```python
from build123d import *

# Parameters (mm, degrees)
SKETCH1_W           = 36
SKETCH1_H           = 55
BOSS_EXTRUDE1_DEPTH = 4
SKETCH2_R           = 1.5
CUT_EXTRUDE1_DEPTH  = 4
FILLET1_R           = 1.5
BOSS_EXTRUDE2_DEPTH = 4


with BuildPart() as part:
    # Sketch1 → Boss-Extrude1 (new body)
    with BuildSketch(Plane.XY):
        Rectangle(SKETCH1_W, SKETCH1_H)
    extrude(amount=BOSS_EXTRUDE1_DEPTH)

    # Sketch2 → Cut-Extrude1 (cut)
    with BuildSketch(Plane.XY.offset(4)):
        with BuildLine():
            Line((-14.75, 23), (-12, 23))
            ThreePointArc((-12, 23), (-10.5, 24.5), (-12, 26))
            Line((-12, 26), (-14.75, 26))
            ThreePointArc((-14.75, 26), (-16.25, 24.5), (-14.75, 23))
        make_face()
        with BuildLine():
            Line((12, 23), (14.75, 23))
            ThreePointArc((14.75, 23), (16.25, 24.5), (14.75, 26))
            Line((14.75, 26), (12, 26))
            ThreePointArc((12, 26), (10.5, 24.5), (12, 23))
        make_face()
        with BuildLine():
            Line((-8, 4), (-7, 4))
            ThreePointArc((-7, 4), (-5.5, 5.5), (-7, 7))
            Line((-7, 7), (-8, 7))
            ThreePointArc((-8, 7), (-9.5, 5.5), (-8, 4))
        make_face()
        with Locations((-2, 5.5)):
            Circle(SKETCH2_R)
        with Locations((2, 5.5)):
            Circle(SKETCH2_R)
        with BuildLine():
            Line((7, 4), (8, 4))
            ThreePointArc((8, 4), (9.5, 5.5), (8, 7))
            Line((8, 7), (7, 7))
            ThreePointArc((7, 7), (5.5, 5.5), (7, 4))
        make_face()
        with BuildLine():
            Line((7, -6), (8, -6))
            ThreePointArc((8, -6), (9.5, -4.5), (8, -3))
            Line((8, -3), (7, -3))
            ThreePointArc((7, -3), (5.5, -4.5), (7, -6))
        make_face()
        with Locations((2, -4.5)):
            Circle(SKETCH2_R)
        with Locations((-2, -4.5)):
            Circle(SKETCH2_R)
        with BuildLine():
            Line((-8, -6), (-7, -6))
            ThreePointArc((-7, -6), (-5.5, -4.5), (-7, -3))
            Line((-7, -3), (-8, -3))
            ThreePointArc((-8, -3), (-9.5, -4.5), (-8, -6))
        make_face()
        with BuildLine():
            Line((-8, -16), (-7, -16))
            ThreePointArc((-7, -16), (-5.5, -14.5), (-7, -13))
            Line((-7, -13), (-8, -13))
            ThreePointArc((-8, -13), (-9.5, -14.5), (-8, -16))
        make_face()
        with BuildLine():
            Line((-8, -26), (-7, -26))
            ThreePointArc((-7, -26), (-5.5, -24.5), (-7, -23))
            Line((-7, -23), (-8, -23))
            ThreePointArc((-8, -23), (-9.5, -24.5), (-8, -26))
        make_face()
        with Locations((-2, -14.5)):
            Circle(SKETCH2_R)
        with Locations((-2, -24.5)):
            Circle(SKETCH2_R)
        with Locations((2, -14.5)):
            Circle(SKETCH2_R)
        with Locations((2, -24.5)):
            Circle(SKETCH2_R)
        with BuildLine():
            Line((7, -26), (8, -26))
            ThreePointArc((8, -26), (9.5, -24.5), (8, -23))
            Line((8, -23), (7, -23))
            ThreePointArc((7, -23), (5.5, -24.5), (7, -26))
        make_face()
        Polygon((-14, 5.5), (-18, 5.5), (-18, -26), (-18, -27.5), (-16.5, -27.5), (-14, -27.5), align=None)
        Polygon((14, 5.5), (14, -27.5), (16.5, -27.5), (18, -27.5), (18, -26), (18, 5.5), align=None)
        with BuildLine():
            ThreePointArc((7, -13), (5.5, -14.5), (7, -16))
            Line((7, -16), (8, -16))
            ThreePointArc((8, -16), (9.5, -14.5), (8, -13))
            Line((8, -13), (7, -13))
        make_face()
    extrude(amount=-CUT_EXTRUDE1_DEPTH, mode=Mode.SUBTRACT)

    # Fillet1
    fillet1_edges = [part.edges().sort_by_distance(p)[0] for p in [
        (18, 5.5, 2),
        (14, -27.5, 2),
        (-14, -27.5, 2),
        (-18, 5.5, 2),
        (-18, 27.5, 2),
        (18, 27.5, 2),
    ]]
    fillet(fillet1_edges, radius=FILLET1_R)

    # Sketch3 → Boss-Extrude2 (add)
    with BuildSketch(Plane.XY.offset(4)):
        with BuildLine():
            Line((-14, 5.5), (-14, 4))
            ThreePointArc((-14, 4), (-14.439339828, 5.060660172), (-15.5, 5.5))
            Line((-15.5, 5.5), (-14, 5.5))
        make_face()
        with BuildLine():
            ThreePointArc((15.5, 5.5), (14.439339828, 5.060660172), (14, 4))
            Line((14, 4), (14, 5.5))
            Line((14, 5.5), (15.5, 5.5))
        make_face()
    extrude(amount=-BOSS_EXTRUDE2_DEPTH)


solid = part.part
```
Geometry: final body of the model. Coordinates: model frame, mm. A direction names the side the tool comes from. Round coordinates to 2 decimals unless told otherwise and drop trailing zeros. Loops run counter-clockwise (first coordinate to the right, second up) from the corner with the lowest first, then second, coordinate; pieces in that order, holes last. Notation, with made-up numbers: (42, -13.75) -> (70, -13.75) arc R23 ccw to (70, -1.75) -> close; hole circle Ø2 at (61, 25.25). An arc over 180 degrees is marked (long way). Use one line per item in the form item = value.
Item 1: Draft query along X for faces 1 (the flat face through (-18, 16, 2)), 2 (the flat face through (-7.5, 4, 2)), 3 (the cylindrical face through (14.45, 5.07, 2.03)), 4 (the flat face through (16, 5.5, 2)). Return one class per face: released by +X, released by -X, zero draft, split by the parting line, or undercut.
Evaluation:
face_1 = released by -X
face_2 = undercut
face_3 = released by +X
face_4 = zero draft
Item 2: Contact query for a flat-ended pin moving along its axis: pin 1 Ø0.5 at (x, z) = (16, 2) entering from -Y. Output: stop coordinate, or through.
Evaluation:
pin_1 = 5.5
Item 3: Material intervals for probe 1 along Y at (x, z) = (7.5, 3.2); probe 2 along Y at (x, z) = (12, 2.05); probe 3 along X at (y, z) = (-5.5, 1.9), sorted ascending.
Evaluation:
probe_1 = -27.5 to -26, -23 to -16, -13 to -6, -3 to 4, 7 to 27.5
probe_2 = -27.5 to 23, 26 to 27.5
probe_3 = -14 to -9.12, -5.88 to -3.12, -0.88 to 0.88, 3.12 to 5.88, 9.12 to 14
Item 4: Access query for faces 5 (the flat face through (7.5, -13, 2)), 6 (the cylindrical face through (13.57, -27.05, 1.97)). Directions: +Z, -Z, +X, -X, +Y, -Y. A direction counts if a zero-diameter tool reaches every point of the face in a straight line with its end or side. Return the directions, or none.
Evaluation:
face_5 = +Z, -Z
face_6 = +Z, -Z, +X, -Y
Item 5: Cut plane A-A on z = 3.1. Give the number of separate pieces and of enclosed holes in the cut face, then the cut area to 3 significant figures.
Evaluation:
separate_pieces = 1
enclosed_holes = 18
area = 1,550 mm2
Item 6: Cut plane B-B on y = 0. Output: boundary loops of the cut face in (x, z).
Evaluation:
outline = (-14, 0) -> (14, 0) -> (14, 4) -> (-14, 4) -> close
